Verification items for this drawing (mm, ordinates from the low corner). A direction names the side the tool comes from. Round coordinates to 2 decimals unless told otherwise and drop trailing zeros. Order: outer loops, then holes, each group sorted by start corner. A loop starts at its lowest first (then second) coordinate and runs counter-clockwise, first axis right, second up.
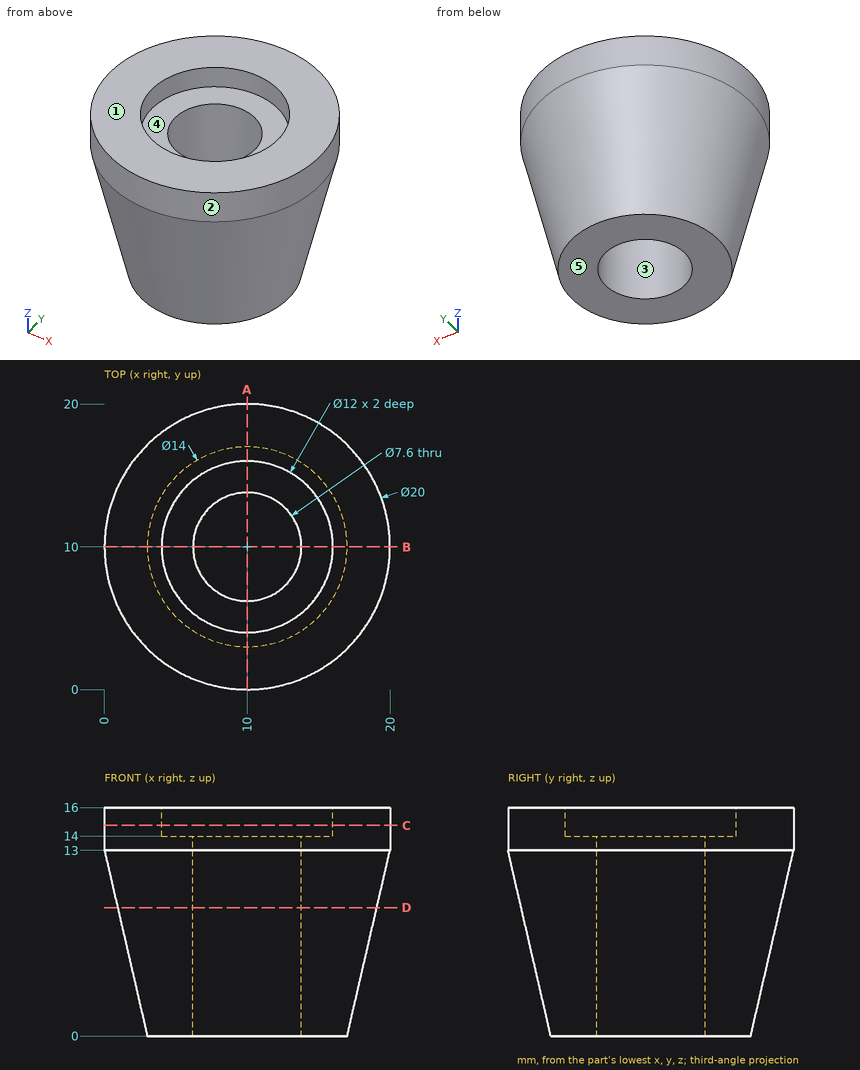
Item 1: Sectioned sample at A-A (x = 10). Record the cut outline in (y, z).
Answer:
outline: (0, 13) - (3, 0) - (6.2, 0) - (6.2, 14) - (4, 14) - (4, 16) - (0, 16) - close; (13.8, 0) - (17, 0) - (20, 13) - (20, 16) - (16, 16) - (16, 14) - (13.8, 14) - close
Item 2: Release check for a two-part mould opening along Y. For the marked faces 1, 2 and 3 record: released by +Y, released by -Y, zero draft, split by the parting line, or undercut.
Answer:
face 1: zero draft
face 2: split by the parting line
face 3: undercut
Item 3: Access from +Z, -Z, +X, -X, +Y, -Y to the whole of each face (thin tool, end or side, straight path). Record for the marked faces 4 and 5.
Answer:
face 4: +Z
face 5: -Z, +X, -X, +Y, -Y
Item 4: Sectioned sample at C-C (z = 14.75). Record the cut outline in (x, y).
Answer:
outline: circle Ø20 at (10, 10); hole circle Ø12 at (10, 10)
Item 5: Scan lines: line 1 along X through (y, z) = (10.5, 7.75); line 2 along Y through (x, z) = (12.75, 12.5); line 3 along Z through (x, y) = (6.5, 12). Record each from-to range of solid material in increasing order.
Answer:
line 1: x = 1.23 to 6.23, 13.77 to 18.77
line 2: y = 0.51 to 7.38, 12.62 to 19.49
line 3: z = 0 to 14
Item 6: Go/stop test with flat-tipped pins: P1, Ø3, axis at y = 7.5, z = 14, coming from the +X side; P2, Ø8, axis at x = 14.5, z = 5.5, coming from the -Y side; P3, Ø4, axis at y = 11, z = 3, coming from the +X side. Record where each tip stops, or that it passes through.
Answer:
P1: stops at x = 19.95
P2: stops at y = 1.23
P3: stops at x = 18.12
Item 7: Sectioned sample at D-D (z = 9). Record the cut outline in (x, y).
Answer:
outline: circle Ø18.15 at (10, 10); hole circle Ø7.6 at (10, 10)
